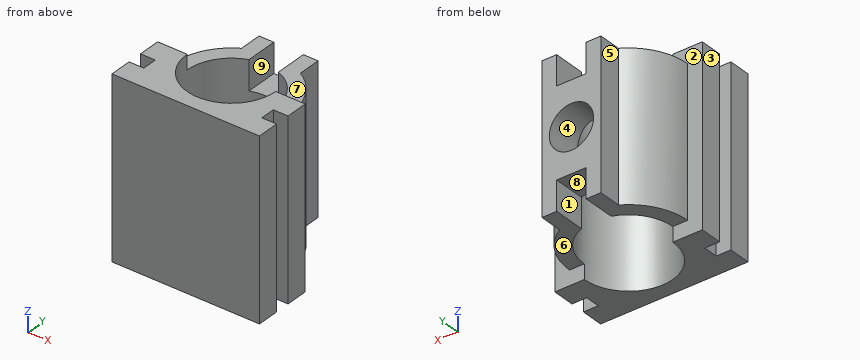
from build123d import *

# Parameters (mm, degrees)
BASE_BLOCK_DEPTH      = 120
BEARING_HOUSING_DEPTH = 100
TOP_SLOTS_SKETCH_W    = 20
TOP_SLOTS_SKETCH_H    = 20
TOP_SLOTS_DEPTH       = 30
TOP_HOLE_SKETCH_R     = 15
TOP_HOLE_30_DEPTH     = 30


with BuildPart() as part:
    # Base Profile Sketch → Base Block (new body)
    with BuildSketch(Plane.XY):
        with BuildLine():
            Line((0, 0), (100, 0))
            Line((100, 0), (100, 15))
            Line((100, 15), (90, 15))
            Line((90, 15), (90, 25))
            Line((90, 25), (100, 25))
            Line((100, 25), (100, 40))
            Line((100, 40), (80, 40))
            ThreePointArc((80, 40), (50, 10), (20, 40))
            Line((20, 40), (0, 40))
            Line((0, 40), (0, 25))
            Line((0, 25), (10, 25))
            Line((10, 25), (10, 15))
            Line((10, 15), (0, 15))
            Line((0, 15), (0, 0))
        make_face()
    extrude(amount=-BASE_BLOCK_DEPTH)

    # Bearing Housing Profile Sketch → Bearing Housing (add)
    with BuildSketch(Plane.XY.offset(-10)):
        with BuildLine():
            ThreePointArc((30, 74.641016151), (15.358983849, 60), (10, 40))
            Line((10, 40), (20, 40))
            ThreePointArc((20, 40), (50, 70), (80, 40))
            Line((80, 40), (90, 40))
            ThreePointArc((90, 40), (84.641016151, 60), (70, 74.641016151))
            ThreePointArc((70, 74.641016151), (50, 80), (30, 74.641016151))
        make_face()
        with BuildLine():
            Line((30, 90), (30, 74.641016151))
            ThreePointArc((30, 74.641016151), (50, 80), (70, 74.641016151))
            Line((70, 74.641016151), (70, 90))
            Line((70, 90), (30, 90))
        make_face()
    extrude(amount=-BEARING_HOUSING_DEPTH)

    # Top Slots Sketch → Top Slots (cut)
    with BuildSketch(Plane(origin=(0, 90, 0), x_dir=(1, 0, 0), z_dir=(0, 1, 0))):
        with Locations((50, 20)):
            Rectangle(TOP_SLOTS_SKETCH_W, TOP_SLOTS_SKETCH_H)
        with Locations((50, 100)):
            Rectangle(TOP_SLOTS_SKETCH_W, TOP_SLOTS_SKETCH_H)
    extrude(amount=-TOP_SLOTS_DEPTH, mode=Mode.SUBTRACT)

    # Top Hole Sketch → Top Hole Ø30 (cut)
    with BuildSketch(Plane(origin=(0, 90, 0), x_dir=(1, 0, 0), z_dir=(0, 1, 0))):
        with Locations(Location((50, 60, 0), (0, 0, 180))):
            Circle(TOP_HOLE_SKETCH_R)
    extrude(amount=-TOP_HOLE_30_DEPTH, mode=Mode.SUBTRACT)


solid = part.part
Source: CAD feature listing. Evaluate the final solid. Frame: model axes, mm. Face numbers are marked on the shaded views. A direction names the side the tool comes from. Coordinates: 2 decimals unless noted, no trailing zeros. Loops run counter-clockwise (first coordinate to the right, second up) from the corner with the lowest first, then second, coordinate; pieces in that order, holes last. Notation, with made-up numbers: (47, 41.25) -> (96, 41.25) arc R27 ccw to (96, 61.25) -> close; hole circle Ø7 at (57.25, -8.75). An arc over 180 degrees is marked (long way). Answer in a Markdown table with one row per item. Add a question column.
Q1. Section B-B on y = 58. Return the cut outline in (x, z).
Q2. Reachability of the marked faces 5, 6, 7, 8 and 9 from +Z, -Z, +X, -X, +Y, -Y: full face, straight path, thin tool, end or side. Return the list, or none.
Q3. Contact query for flat-ended pins moving along their axis: pin 1 Ø6 at (x, z) = (10.5, -44.5) entering from +Y; pin 2 Ø6 at (y, z) = (75, -16.5) entering from -X; pin 3 Ø1.5 at (y, z) = (52.5, -64) entering from -X. Output: stop coordinate, or through.
Q4. Pull-direction query (X, two-part tool) for the marked faces 1, 2, 3 and 4; classes: pulls with the +X half, pulls with the -X half, needs draft (parallel to the pull), parting line crosses it, or undercut.
Q5. Section D-D on z = -60. Return the cut outline in (x, y), and give its area (3 significant figures).
Q6. Ray query, line 1 along Y through (x, z) = (6, -101); line 2 along X through (y, z) = (83.5, -28.5); line 3 along X through (y, z) = (81, -60). Return the intervals inside material, ascending.
Q7. Section C-C on z = -79.5. Return the cut outline in (x, y).
Q8. Section A-A on x = 50. Return the cut outline in (y, z).
Computed values:
| question | item | result |
|---|---|---|
| 1 | outline | (14.28, -110) -> (26, -110) -> (26, -10) -> (14.28, -10) -> close; (74, -110) -> (85.72, -110) -> (85.72, -10) -> (74, -10) -> close |
| 2 | face 5 | +Z, -Z, -X, +Y |
| 2 | face 6 | -Z, +X, -X, +Y |
| 2 | face 7 | +Z, +X, -X, +Y |
| 2 | face 8 | -Z, +Y |
| 2 | face 9 | +Z, +Y |
| 3 | pin 1 | stops at y = 56.36 |
| 3 | pin 2 | stops at x = 26 |
| 3 | pin 3 | stops at x = 11.76 |
| 4 | face 1 | undercut |
| 4 | face 2 | needs draft |
| 4 | face 3 | pulls with the -X half |
| 4 | face 4 | undercut |
| 5 | outline | (0, 0) -> (100, 0) -> (100, 15) -> (90, 15) -> (90, 25) -> (100, 25) -> (100, 40) -> (90, 40) arc R40 ccw to (70, 74.64) -> (70, 90) -> (65, 90) -> (65, 65.98) arc R30 cw (long way) to (35, 65.98) -> (35, 90) -> (30, 90) -> (30, 74.64) arc R40 ccw to (10, 40) -> (0, 40) -> (0, 25) -> (10, 25) -> (10, 15) -> (0, 15) -> close |
| 5 | area | 3,320 mm^2 |
| 6 | line 1 | y = 0 to 15, 25 to 40 |
| 6 | line 2 | x = 30 to 40, 60 to 70 |
| 6 | line 3 | x = 30 to 35, 65 to 70 |
| 7 | outline | (0, 0) -> (100, 0) -> (100, 15) -> (90, 15) -> (90, 25) -> (100, 25) -> (100, 40) -> (90, 40) arc R40 ccw to (70, 74.64) -> (70, 90) -> (30, 90) -> (30, 74.64) arc R40 ccw to (10, 40) -> (0, 40) -> (0, 25) -> (10, 25) -> (10, 15) -> (0, 15) -> close; hole circle Ø60 at (50, 40) |
| 8 | outline | (0, -120) -> (10, -120) -> (10, 0) -> (0, 0) -> close; (70, -90) -> (90, -90) -> (90, -75) -> (70, -75) -> close; (70, -45) -> (90, -45) -> (90, -30) -> (70, -30) -> close |
